Geometry: see drawing. Coordinates: mm, zero at the bounding-box minimum. A direction names the side the tool comes from. Round coordinates to 2 decimals unless told otherwise and drop trailing zeros. Loops run counter-clockwise (first coordinate to the right, second up) from the corner with the lowest first, then second, coordinate; pieces in that order, holes last. Notation, with made-up numbers: (-33, 79.5) - (16, 79.5) arc R12 ccw to (16, 93.5) - close; hole circle Ø5 at (-8, -10.75). An arc over 180 degrees is marked (long way). Answer in a Markdown table with one row per item. Add a question column.
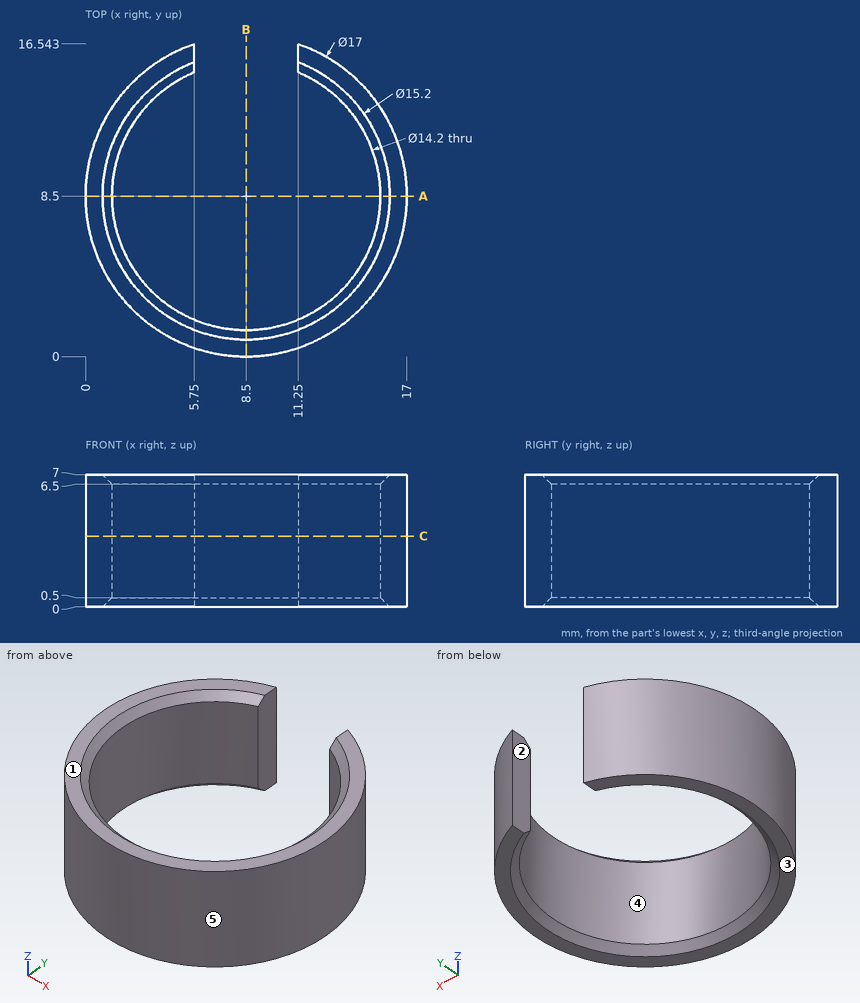
1) Section B-B, the plane x = 8.5. Return the cut outline in (y, z).
2) Section C-C, the plane z = 3.75. Return the cut outline in (x, y).
3) Material intervals for line 1 along X through (y, z) = (8.5, 3.55); line 2 along Y through (x, z) = (8.5, 3.6); line 3 along X through (y, z) = (9.75, 1.25), sorted ascending. Write a range as from..to.
4) Contact query for flat-ended pins moving along their axis: pin 1 Ø6 at (x, y) = (10.5, 9.5) entering from -Z; pin 2 Ø0.7 at (y, z) = (16, 2.5) entering from -X; pin 3 Ø4 at (x, y) = (2.5, 12.5) entering from +Z; pin 4 Ø1 at (y, z) = (12.5, 1.5) entering from -X. Output: stop coordinate, or through.
5) Pull-direction query (X, two-part tool) for the marked faces 3, 4 and 5; classes: pulls with the +X half, pulls with the -X half, needs draft (parallel to the pull), parting line crosses it, or undercut.
6) Reachability of the marked faces 1 and 2 from +Z, -Z, +X, -X, +Y, -Y: full face, straight path, thin tool, end or side. Return the list, or none.
7) Section A-A, the plane y = 8.5. Return the cut outline in (x, z), and give its area (3 significant figures).
Evaluation:
| question | item | result |
|---|---|---|
| 1 | outline | (0, 0) - (0.9, 0) - (1.4, 0.5) - (1.4, 6.5) - (0.9, 7) - (0, 7) - close |
| 2 | outline | (5.75, 15.05) - (5.75, 16.54) arc R8.5 ccw (long way) to (11.25, 16.54) - (11.25, 15.05) arc R7.1 cw (long way) to start |
| 3 | line 1 | x = 0..1.4, 15.6..17 |
| 3 | line 2 | y = 0..1.4 |
| 3 | line 3 | x = 0.09..1.51, 15.49..16.91 |
| 4 | pin 1 | passes through |
| 4 | pin 2 | stops at x = 3.9 |
| 4 | pin 3 | stops at z = 7 |
| 4 | pin 4 | stops at x = 0.75 |
| 5 | face 3 | needs draft |
| 5 | face 4 | undercut |
| 5 | face 5 | parting line crosses it |
| 6 | face 1 | +Z, +X, -X, +Y, -Y |
| 6 | face 2 | +Z, -Z, +Y |
| 7 | outline | (0, 0) - (0.9, 0) - (1.4, 0.5) - (1.4, 6.5) - (0.9, 7) - (0, 7) - close; (15.6, 0.5) - (16.1, 0) - (17, 0) - (17, 7) - (16.1, 7) - (15.6, 6.5) - close |
| 7 | area | 19.1 mm² |
